The listing builds one solid part. Answer for the finished solid, in the listing's coordinates (mm). Face numbers are marked on the shaded views. A direction names the side the tool comes from. Give positions to 0.01 mm unless a question says otherwise; leave off trailing zeros. Order: outer loops, then holes, each group sorted by start corner. A loop starts at its lowest first (then second) coordinate and runs counter-clockwise, first axis right, second up. Notation, with made-up numbers: M -10.75,84.5 L 34.25,84.5 A7 ccw 34.25,94.5 Z; hole C 85,-12.5 d1. An arc over 180 degrees is marked long. Answer as a JSON object with one key per item and string values. Group by question number.
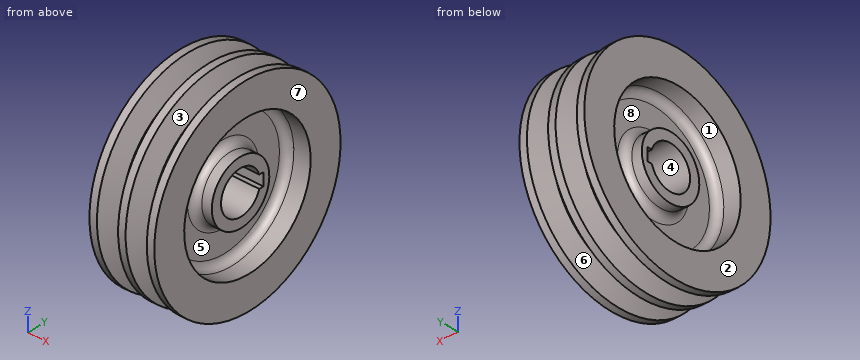
```python
from build123d import *

# Parameters (mm, degrees)
FRONT_RECESS_110_SKETCH_R    = 55
FRONT_RECESS_110_DEPTH       = 19.5
REAR_START                   = -19.5
REAR_RECESS_110_SKETCH_R     = 55
REAR_RECESS_110_DEPTH        = 19.5
FRONT_HUB_50_SKETCH_R        = 25
FRONT_HUB_50_DEPTH           = 14
REAR_START_2                 = 14
REAR_HUB_50_SKETCH_R         = 25
REAR_HUB_50_DEPTH            = 14
KEYED_BORE_20_DEPTH          = 89
FRONT_RECESS_RIM_FILLET_R6_R = 6
REAR_RECESS_RIM_FILLET_R6_R  = 6
FRONT_HUB_ROOT_FILLET_R6_R   = 6
REAR_HUB_ROOT_FILLET_R6_R    = 6


with BuildPart() as part:
    # Pulley Rim Profile Sketch → Twin Groove Pulley Body (revolve)
    with BuildSketch(Plane.XY, mode=Mode.PRIVATE) as twin_groove_pulley_body_sk:
        Polygon((52, 0), (0, 0), (0, 81), (6, 81), (10.969940868, 64.744055898), (18.030059132, 64.744055898), (23, 81), (29, 81), (33.969940868, 64.744055898), (41.030059132, 64.744055898), (46, 81), (52, 81), align=None)
    revolve(twin_groove_pulley_body_sk.sketch.rotate(Axis((52, 0, 0), (-1, 0, 0)), 90), axis=Axis((52, 0, 0), (-1, 0, 0)))

    # Front Recess Ø110 Sketch → Front Recess Ø110 (cut)
    with BuildSketch(Plane(origin=(52, 0, 0), x_dir=(0, 0, -1), z_dir=(1, 0, 0))):
        Circle(FRONT_RECESS_110_SKETCH_R)
    extrude(amount=-FRONT_RECESS_110_DEPTH, mode=Mode.SUBTRACT)

    # Rear Recess Ø110 Sketch → Rear Recess Ø110 (cut)
    with BuildSketch(Plane.ZY.offset(REAR_START)):
        with Locations(Location((0, 0, 0), (0, 0, 180))):
            Circle(REAR_RECESS_110_SKETCH_R)
    extrude(amount=REAR_RECESS_110_DEPTH, mode=Mode.SUBTRACT)

    # Front Hub Ø50 Sketch → Front Hub Ø50 (add)
    with BuildSketch(Plane(origin=(32.5, 0, 0), x_dir=(0, 0, -1), z_dir=(1, 0, 0))):
        Circle(FRONT_HUB_50_SKETCH_R)
    extrude(amount=FRONT_HUB_50_DEPTH)

    # Rear Hub Ø50 Sketch → Rear Hub Ø50 (add)
    with BuildSketch(Plane.ZY.offset(-19.5).offset(REAR_START_2)):
        with Locations(Location((0, 0, 0), (0, 0, 180))):
            Circle(REAR_HUB_50_SKETCH_R)
    extrude(amount=-REAR_HUB_50_DEPTH)

    # Keyed Bore Ø20 Sketch → Keyed Bore Ø20 (cut)
    with BuildSketch(Plane.ZY.offset(-5.5)):
        with BuildLine():
            Line((0, 20), (5, 20))
            Line((5, 20), (5, 16.248076809))
            ThreePointArc((5, 16.248076809), (0, -17), (-5, 16.248076809))
            Line((-5, 16.248076809), (-5, 20))
            Line((-5, 20), (0, 20))
        make_face()
    extrude(amount=-KEYED_BORE_20_DEPTH, mode=Mode.SUBTRACT)

    # Front Recess Rim Fillet R6
    front_recess_rim_fillet_r6_edges = [part.edges().sort_by_distance(p)[0] for p in [
        (32.5, 0, 55),
    ]]
    fillet(front_recess_rim_fillet_r6_edges, radius=FRONT_RECESS_RIM_FILLET_R6_R)

    # Rear Recess Rim Fillet R6
    rear_recess_rim_fillet_r6_edges = [part.edges().sort_by_distance(p)[0] for p in [
        (19.5, 0, 55),
    ]]
    fillet(rear_recess_rim_fillet_r6_edges, radius=REAR_RECESS_RIM_FILLET_R6_R)

    # Front Hub Root Fillet R6
    front_hub_root_fillet_r6_edges = [part.edges().sort_by_distance(p)[0] for p in [
        (32.5, 0, 25),
    ]]
    fillet(front_hub_root_fillet_r6_edges, radius=FRONT_HUB_ROOT_FILLET_R6_R)

    # Rear Hub Root Fillet R6
    rear_hub_root_fillet_r6_edges = [part.edges().sort_by_distance(p)[0] for p in [
        (19.5, 0, 25),
    ]]
    fillet(rear_hub_root_fillet_r6_edges, radius=REAR_HUB_ROOT_FILLET_R6_R)


solid = part.part
```
Item 1: A tool of negligible diameter and unlimited length cuts with its end or side. For the marked faces 1, 2, 3, 4 and 5, from which of +Z, -Z, +X, -X, +Y, -Y can it reach the whole face along a straight path? Write none if from no direction.
Item 2: Section A-A (x = 27) is taken. Determine the outline of the cut face in (y, z).
Item 3: Consider probe 1 along X at (y, z) = (-24, -63); probe 2 along X at (y, z) = (19.5, 64); probe 3 along Y at (x, z) = (49, 0). Determine where each line is inside the solid, lowest interval first. Write a range as from..to.
Item 4: Flat-ended cylindrical pins translate along their axes: P1, Ø3, axis at x = 39.5, z = -40, coming from the -Y side; P2, Ø4, axis at x = 36, y = 18, coming from the -Z side; P3, Ø2, axis at x = 15.5, y = -25, coming from the -Z side. Find the tip coordinate at first contact, or state that the pin passes through.
Item 5: Section B-B (x = 48.5) is taken. Determine the outline of the cut face in (y, z), and give its area (3 significant figures).
Item 6: Determine the mould class of the marked faces 6, 7 and 8 for opening direction Y: released by +Y, released by -Y, zero draft, split by the parting line, or undercut.
Values found:
{
 "1": {"face 1": "-X", "face 2": "+Z, -Z, -X, +Y, -Y", "face 3": "none", "face 4": "+X, -X", "face 5": "+X"},
 "2": {"outline": "C 0,0 d162; hole M 16.25,-5 L 20,-5 L 20,5 L 16.25,5 A17 ccw long Z"},
 "3": {"probe 1": "x = 0..10.15, 18.85..33.15, 41.85..52", "probe 2": "x = 0..10.31, 18.69..33.31, 41.69..52", "probe 3": "y = -81..-55, 55..81"},
 "4": {"P1": "stops at y = -52.05", "P2": "stops at z = -62.74", "P3": "stops at z = -60.13"},
 "5": {"outline": "C 0,0 d162; hole C 0,0 d110", "area": "11,100 mm^2"},
 "6": {"face 6": "split by the parting line", "face 7": "zero draft", "face 8": "undercut"}
}
